Input: part model. Units: mm. Frame: model coordinates. A direction names the side the tool comes from. Coordinates: 2 decimals unless noted, no trailing zeros. Write each loop counter-clockwise with the first axis right and the second up, starting at its lowest first coordinate (ties: lowest second). Pieces come first, ordered by that corner, then holes. Notation, with made-up numbers: M -16.5,-35 L -1.5,-35 A28 cw -1.5,-3 Z; hole C -10,40 d2. An arc over 180 degrees is marked long. Use one line per item in the form item = value.
from build123d import *

# Parameters (mm, degrees)
SKETCH1_W           = 400
SKETCH1_H           = 230
BOSS_EXTRUDE1_DEPTH = 10
SKETCH2_R           = 4.5
CUT_EXTRUDE1_DEPTH  = 25
SKETCH3_R           = 6.5
CUT_EXTRUDE2_DEPTH  = 9


with BuildPart() as part:
    # Sketch1 → Boss-Extrude1 (new body)
    with BuildSketch(Plane.XY):
        Rectangle(SKETCH1_W, SKETCH1_H)
    extrude(amount=BOSS_EXTRUDE1_DEPTH)

    # Sketch2 → Cut-Extrude1 (cut)
    with BuildSketch(Plane(origin=(0, 0, 0), x_dir=(-1, 0, 0), z_dir=(0, 0, -1))):
        with Locations((192.5, -85)):
            Circle(SKETCH2_R)
        with Locations((192.5, 0)):
            Circle(SKETCH2_R)
        with Locations((192.5, 85)):
            Circle(SKETCH2_R)
    cut_extrude1 = extrude(amount=-CUT_EXTRUDE1_DEPTH, mode=Mode.SUBTRACT)

    # Sketch3 → Cut-Extrude2 (cut)
    with BuildSketch(Plane(origin=(0, 0, 0), x_dir=(-1, 0, 0), z_dir=(0, 0, -1))):
        with Locations((192.5, -85)):
            Circle(SKETCH3_R)
        with Locations((192.5, 0)):
            Circle(SKETCH3_R)
        with Locations((192.5, 85)):
            Circle(SKETCH3_R)
    cut_extrude2 = extrude(amount=-CUT_EXTRUDE2_DEPTH, mode=Mode.SUBTRACT)

    # Mirror1: Cut-Extrude1, Cut-Extrude2 across plane
    add(cut_extrude1.mirror(Plane(origin=(0, 0, 0), x_dir=(0, 0, 1), z_dir=(1, 0, 0))), mode=Mode.SUBTRACT)
    add(cut_extrude2.mirror(Plane(origin=(0, 0, 0), x_dir=(0, 0, 1), z_dir=(1, 0, 0))), mode=Mode.SUBTRACT)


solid = part.part
(1) Set-up query: faces 1 (the flat face through (-197, 2, 9)), 2 (the cylindrical face through (196.792, 86.352, 9.493)). Return all of +Z, -Z, +X, -X, +Y, -Y with unobstructed straight access to the full face (end or side cutting, diameter ignored); none if empty.
Computed:
face_1 = -Z
face_2 = +Z, -Z
(2) Pull-direction query (X, two-part tool) for faces 3 (the flat face through (-200, -2, 5)), 4 (the flat face through (-3, 2, 0)), 5 (the cylindrical face through (-186, 0, 4)); classes: pulls with the +X half, pulls with the -X half, needs draft (parallel to the pull), parting line crosses it, or undercut.
Computed:
face_3 = pulls with the -X half
face_4 = needs draft
face_5 = undercut
(3) Section query A-A on y = 85. Return the cut outline in (x, z), plus the area to 3 significant figures.
Computed:
outline = M -200,0 L -199,0 L -199,9 L -197,9 L -197,10 L -200,10 Z; M -188,9 L -186,9 L -186,0 L 186,0 L 186,9 L 188,9 L 188,10 L -188,10 Z; M 197,9 L 199,9 L 199,0 L 200,0 L 200,10 L 197,10 Z
area = 3,750 mm^2
(4) Section query B-B on x = -192.5. Return the cut outline in (y, z), plus the area to 3 significant figures.
Computed:
outline = M -115,0 L -91.5,0 L -91.5,9 L -89.5,9 L -89.5,10 L -115,10 Z; M -80.5,9 L -78.5,9 L -78.5,0 L -6.5,0 L -6.5,9 L -4.5,9 L -4.5,10 L -80.5,10 Z; M 4.5,9 L 6.5,9 L 6.5,0 L 78.5,0 L 78.5,9 L 80.5,9 L 80.5,10 L 4.5,10 Z; M 89.5,9 L 91.5,9 L 91.5,0 L 115,0 L 115,10 L 89.5,10 Z
area = 1,920 mm^2
(5) Line query: probe 1 along Y at (x, z) = (192.5, 5.5); probe 2 along Y at (x, z) = (-192.5, 9.65); probe 3 along X at (y, z) = (-86, 3.25). Output: solid intervals per line, ascending.
Computed:
probe_1 = -115 to -91.5, -78.5 to -6.5, 6.5 to 78.5, 91.5 to 115
probe_2 = -115 to -89.5, -80.5 to -4.5, 4.5 to 80.5, 89.5 to 115
probe_3 = -200 to -198.92, -186.08 to 186.08, 198.92 to 200
(6) First-contact query: pin 1 Ø10.5 at (x, y) = (-192.5, 85) entering from -Z; pin 2 Ø14.5 at (x, y) = (-192.5, 85.5) entering from -Z. Flat tips, straight axial feed; report the tip coordinate or a pass-through.
Computed:
pin_1 = 9
pin_2 = 0
